Design review of the part built by this model. Coordinates are the model's own, in mm. A direction names the side the tool comes from. Give positions to 0.01 mm unless a question says otherwise; leave off trailing zeros. Loops run counter-clockwise (first coordinate to the right, second up) from the corner with the lowest first, then second, coordinate; pieces in that order, holes last. Notation, with made-up numbers: M 65.5,38 L 89.5,38 A20 ccw 89.5,48 Z; hole C -16.5,-38 d4. An arc over 180 degrees is marked long. Use a Markdown table: item, result. Add a question column.
(1) Draft analysis for pull direction Y (two halves, no side actions). For faces 1 (the face through (8, -9, 38)), 2 (the face through (2.38, -10.74, 18.49)), 3 (the face through (-9.05, -15.56, 21.27)), state which applies: pulls with the +Y half, pulls with the -Y half, needs draft (parallel to the pull), parting line crosses it, or undercut.
(2) Add section B-B, the plane x = 12.5. Give the boundary of the cut face in (y, z).
(3) For faces 4 (the face through (-8.3, -16.2, 5)), 5 (the face through (-8.95, 15.62, 21.27)), 6 (the face through (8.95, -15.62, 21.27)), list the 3-axis set-ups (+Z, -Z, +X, -X, +Y, -Y) from which the entire face can be reached by the end or side of a thin tool; tool diameter is ignored.
(4) Add section A-A, the plane z = 20.5. Give the boundary of the cut face in (x, y), then the cut area to 3 significant figures.
(5) Add section C-C, the plane y = 0. Give the boundary of the cut face in (x, z).
(6) Insertion check: pin 1 Ø4 at (x, z) = (-8, 12) entering from +Y; pin 2 Ø1.5 at (y, z) = (0.5, 13.5) entering from -X; pin 3 Ø12 at (x, z) = (9.5, 15.5) entering from +Y. Each pin has a flat end and moves straight along its axis. Give the tip position at first contact, or say it passes through.
(7) Add section D-D, the plane y = -17.5. Give the boundary of the cut face in (x, z).
(8) For probe 1 along Z at (x, y) = (-7, -18); probe 2 along Y at (x, z) = (0, 11); probe 3 along Y at (x, z) = (0.5, 24), list the stretches that pass through material, from the lowest coordinate up.
```python
from build123d import *

# Parameters (mm, degrees)
SKETCH1_R                  = 22
BOSS_EXTRUDE_DEPTH         = 5
BOSS_EXTRUDE1_DEPTH        = 33
M24X2_0_TAPPED_HOLE1_D     = 22
M24X2_0_TAPPED_HOLE1_DEPTH = 58
M24X2_0_TAPPED_HOLE1_TIP   = 6.609466809
CHAMFER2_SIZE              = 0.5


with BuildPart() as part:
    # Sketch1 → Boss-Extrude (new body)
    with BuildSketch(Plane.XY):
        Circle(SKETCH1_R)
    extrude(amount=BOSS_EXTRUDE_DEPTH)

    # Sketch2 → Boss-Extrude1 (add)
    with BuildSketch(Plane.XY.offset(5)):
        Polygon((-17.945989557, -10.485297269), (0.107539023, -20.784331487), (18.05352858, -10.299034218), (17.945989557, 10.485297269), (-0.107539023, 20.784331487), (-18.05352858, 10.299034218), align=None)
    extrude(amount=BOSS_EXTRUDE1_DEPTH)

    # Sketch4 → Cut-Revolve1 (revolve, cut)
    with BuildSketch(Plane(origin=(0, 0, 0), x_dir=(0, 0, -1), z_dir=(1, 0, 0)), mode=Mode.PRIVATE) as cut_revolve1_sk:
        Polygon((-8.577004511, -2.997330388), (-6.875334866, -5.94470867), (-8.577004511, -5.94470867), align=None)
    revolve(cut_revolve1_sk.sketch.rotate(Axis((0, 0, 0), (0, 0, 1)), 270), axis=Axis((0, 0, 0), (0, 0, 1)), mode=Mode.SUBTRACT)

    # M24x2.0 Tapped Hole1
    with Locations(Plane.XY.offset(38)):
        with Locations((0, 0)):
            Hole(M24X2_0_TAPPED_HOLE1_D / 2, depth=M24X2_0_TAPPED_HOLE1_DEPTH)
            with Locations((0, 0, -(M24X2_0_TAPPED_HOLE1_DEPTH + M24X2_0_TAPPED_HOLE1_TIP / 2))):  # 118° drill point
                Cone(0, M24X2_0_TAPPED_HOLE1_D / 2, M24X2_0_TAPPED_HOLE1_TIP, mode=Mode.SUBTRACT)

    # Chamfer2
    chamfer2_edges = [part.edges().sort_by_distance(p)[0] for p in [
        (11, 0, 38),
    ]]
    chamfer(chamfer2_edges, length=CHAMFER2_SIZE)


solid = part.part
```
Established:
| question | item | result |
|---|---|---|
| 1 | face 1 | needs draft |
| 1 | face 2 | undercut |
| 1 | face 3 | pulls with the -Y half |
| 2 | outline | M -18.1,0 L 18.1,0 L 18.1,5 L 13.59,5 L 13.59,38 L -13.54,38 L -13.54,5 L -18.1,5 Z |
| 3 | face 4 | +Z |
| 3 | face 5 | +Z, -X, +Y |
| 3 | face 6 | +Z, +X, -Y |
| 4 | outline | M -18.05,10.3 L -17.95,-10.49 L 0.11,-20.78 L 18.05,-10.3 L 17.95,10.49 L -0.11,20.78 Z; hole C 0,0 d22 |
| 4 | area | 742 mm^2 |
| 5 | outline | M -22,0 L -11,0 L -11,37.5 L -11.5,38 L -18,38 L -18,5 L -22,5 Z; M 11,0 L 22,0 L 22,5 L 18,5 L 18,38 L 11.5,38 L 11,37.5 Z |
| 6 | pin 1 | y = 17.34 |
| 6 | pin 2 | x = -18.01 |
| 6 | pin 3 | y = 18.73 |
| 7 | outline | M -13.33,0 L 13.33,0 L 13.33,5 L 5.73,5 L 5.73,38 L -5.65,38 L -5.65,5 L -13.33,5 Z |
| 8 | probe 1 | 0 to 5 |
| 8 | probe 2 | -20.72 to -11, 11 to 20.72 |
| 8 | probe 3 | -20.56 to -10.99, 10.99 to 20.44 |
